Check sheet for the drawn part. Datum: minimum x, y, z corner. Units: mm. A direction names the side the tool comes from. Give positions to 0.01 mm unless a question says otherwise; leave off trailing zeros. Loops run counter-clockwise (first coordinate to the right, second up) from the corner with the lowest first, then second, coordinate; pieces in that order, holes last. Notation, with made-up numbers: (86, 0.25) - (121, 0.25) arc R10 cw to (121, 17.25) - close; hole circle Ø1 at (33.5, 85). An arc over 180 degrees is marked (long way). Use one line per item in the form item = value.
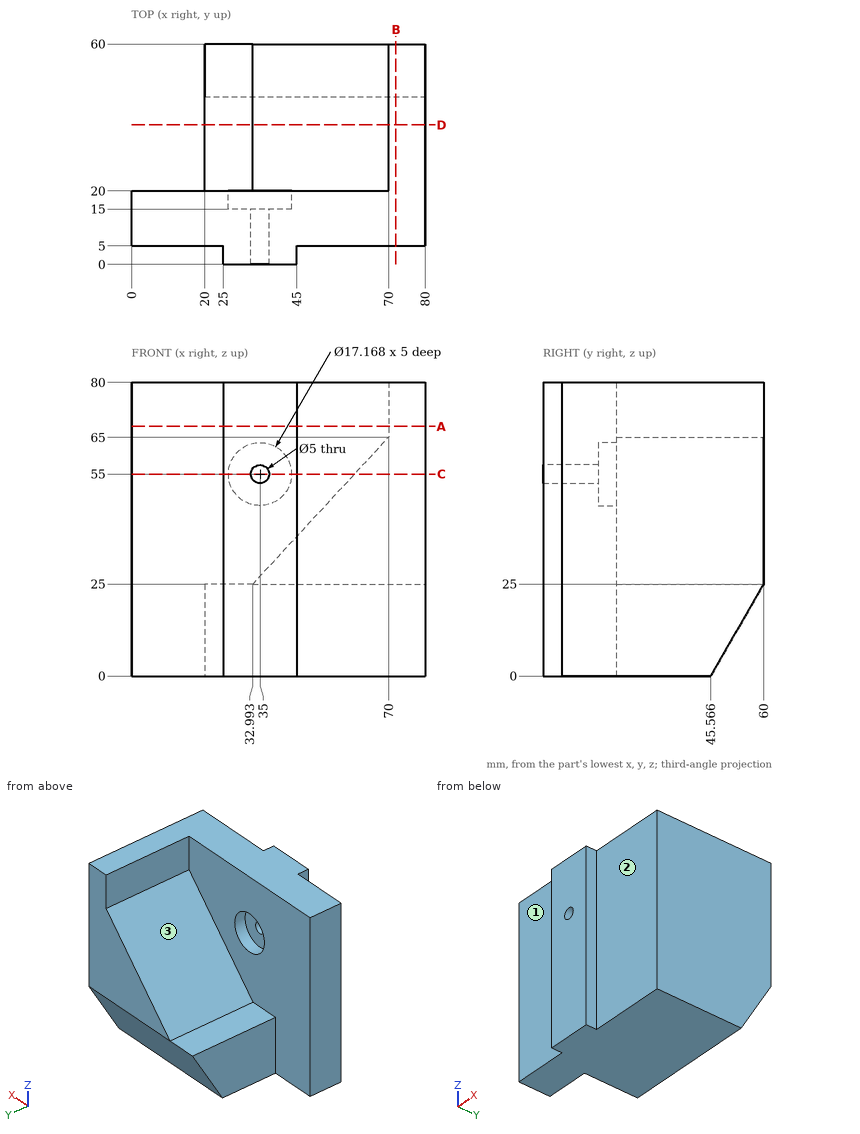
1. Section check B-B, the plane x = 72. Record the cut outline in (y, z).
Result set:
outline = (5, 0) - (45.57, 0) - (60, 25) - (60, 80) - (5, 80) - close
2. Section check C-C, the plane z = 55. Record the cut outline in (x, y), then the cut area to 3 significant figures.
Result set:
outline = (0, 5) - (25, 5) - (25, 0) - (32.5, 0) - (32.5, 15) - (26.42, 15) - (26.42, 20) - (0, 20) - close; (37.5, 0) - (45, 0) - (45, 5) - (80, 5) - (80, 60) - (60.75, 60) - (60.75, 20) - (43.58, 20) - (43.58, 15) - (37.5, 15) - close
area = 1,910 mm²
3. Section check D-D, the plane y = 38. Record the cut outline in (x, z).
Result set:
outline = (20, 0) - (80, 0) - (80, 80) - (70, 80) - (70, 65) - (32.99, 25) - (20, 25) - close
4. Section check A-A, the plane z = 68. Record the cut outline in (x, y), then the cut area to 3 significant figures.
Result set:
outline = (0, 5) - (25, 5) - (25, 0) - (45, 0) - (45, 5) - (80, 5) - (80, 60) - (70, 60) - (70, 20) - (0, 20) - close
area = 1,700 mm²
5. Scan lines: probe 1 along X at (y, z) = (18.6, 55); probe 2 along X at (y, z) = (7.25, 55); probe 3 along Y at (x, z) = (21, 75.5). Record each from-to range of solid material in increasing order.
Result set:
probe_1 = 0 to 26.42, 43.58 to 80
probe_2 = 0 to 32.5, 37.5 to 80
probe_3 = 5 to 20
6. Tool access check on the marked faces 1, 2 and 3. Record the directions out of +Z, -Z, +X, -X, +Y, -Y that give a thin tool (end or side, any length) a straight path to the whole face; none if there is none.
Result set:
face_1 = +Z, -Z, -X, -Y
face_2 = +Z, -Z, +X, -Y
face_3 = +Z, -X, +Y
7. Depth check by flat-ended pin: pin 1 Ø12 at (y, z) = (49, 71.5) entering from -X; pin 2 Ø1 at (x, z) = (55, 19.5) entering from -Y; pin 3 Ø5.5 at (y, z) = (2, 45.5) entering from +X. Enter the tip coordinate at first touch or a pass-through.
Result set:
pin_1 = 70
pin_2 = 5
pin_3 = 45
